Can you work these out from the model? Positions are in its coordinate system, mm. A direction names the side the tool comes from. Give positions to 0.01 mm unless a question says otherwise; leave off trailing zeros. Loops run counter-clockwise (first coordinate to the right, second up) from the corner with the lowest first, then second, coordinate; pieces in that order, holes last. Notation, with made-up numbers: (-11, 86) -> (28, 86) arc R18 cw to (28, 106) -> close; hole circle Ø3 at (-29, 49.25). An arc over 180 degrees is marked (long way). Return JSON: item names as keys, results as strings. Group by question number.
Q1. I need wall thicknesses on line 1 along Y through (x, z) = (-30, 0); line 2 along Y through (x, z) = (0, 11); line 3 along X through (y, z) = (-58, 2.5). Which ranges of each line are inside material? Lowest first, please. Write a range as [from, to].
Q2. Suppose I cut it at D-D, the plane y = -55. Please give me the cut outline in (x, z).
Q3. Will these pins go through, and if not, where does the flat tip stop? pin 1 (5 mm diameter, centred on x = -32, y = 23.5, fed in from -Z); pin 2 (1.5 mm diameter, centred on x = 6, z = 5.5, fed in from -Y); pin 3 (10 mm diameter, centred on y = 70.5, z = -10, fed in from -X); pin 4 (3 mm diameter, centred on y = 9, z = 6.5, fed in from +X).
Q4. Thinking about a two-plate mould opening in X: for faces 1 (the flat face through (19, -19, 4)), 2 (the cylindrical face through (41.53, -79.845, 0.056)), 3 (the cylindrical face through (-12.831, -46.555, 0.056)), which applies, pulls with the +X half, pulls with the -X half, needs draft (parallel to the pull), parting line crosses it, or undercut?
Q5. Suppose I cut it at A-A, the plane y = 0. Please give me the cut outline in (x, z).
Q6. Suppose I cut it at C-C, the plane x = 39.5. Please give me the cut outline in (y, z).
Q7. Which directions (+Z, -Z, +X, -X, +Y, -Y) give clear straight access to the entire face, cutting with the end or side of a thin tool? Please do faces 4 (the flat face through (0, -11, -22)), 5 (the cylindrical face through (23.846, 7.509, -12.874)), 6 (the cylindrical face through (23.846, 7.509, 13.126)).
Q8. Suppose I cut it at B-B, the plane x = 0. Please give me the cut outline in (y, z).
```python
from build123d import *

# Parameters (mm, degrees)
SKETCH_1_R          = 90
SKETCH_1_R_2        = 10.1
EXTRUDE_1_DEPTH     = 4
SKETCH_2_R          = 25
SKETCH_2_R_2        = 10.1
EXTRUDE_2_DEPTH     = 22
SKETCH_3_R          = 18
CUT_EXTRUDE_1_DEPTH = 30


with BuildPart() as part:
    # 草图1 → 凸台-拉伸1 (new, symmetric)
    with BuildSketch(Plane.XY):
        Circle(SKETCH_1_R)
        Circle(SKETCH_1_R_2, mode=Mode.SUBTRACT)
    extrude(amount=EXTRUDE_1_DEPTH, both=True)

    # 草图2 → 凸台-拉伸2 (add, symmetric)
    with BuildSketch(Plane.XY):
        Circle(SKETCH_2_R)
        Circle(SKETCH_2_R_2, mode=Mode.SUBTRACT)
    extrude(amount=EXTRUDE_2_DEPTH, both=True)

    # 草图3 → 切除-拉伸1 (cut, symmetric)
    with BuildSketch(Plane.XY):
        with Locations((60, 0)):
            Circle(SKETCH_3_R)
        with Locations((30, 51.961524227)):
            Circle(SKETCH_3_R)
        with Locations((-30, 51.961524227)):
            Circle(SKETCH_3_R)
        with Locations((-60, 0)):
            Circle(SKETCH_3_R)
        with Locations((-30, -51.961524227)):
            Circle(SKETCH_3_R)
        with Locations((30, -51.961524227)):
            Circle(SKETCH_3_R)
    extrude(amount=CUT_EXTRUDE_1_DEPTH, both=True, mode=Mode.SUBTRACT)


solid = part.part
```
Ans:
{
 "1": {"line 1": "y = [-84.85, -69.96], [-33.96, 33.96], [69.96, 84.85]", "line 2": "y = [-25, -10.1], [10.1, 25]", "line 3": "x = [-68.82, -46.96], [-13.04, 13.04], [46.96, 68.82]"},
 "2": {"outline": "(-71.24, -4) -> (-47.74, -4) -> (-47.74, 4) -> (-71.24, 4) -> close; (-12.26, -4) -> (12.26, -4) -> (12.26, 4) -> (-12.26, 4) -> close; (47.74, -4) -> (71.24, -4) -> (71.24, 4) -> (47.74, 4) -> close"},
 "3": {"pin 1": "stops at z = -4", "pin 2": "stops at y = -24.44", "pin 3": "passes through", "pin 4": "stops at x = 23.85"},
 "4": {"face 1": "needs draft", "face 2": "parting line crosses it", "face 3": "undercut"},
 "5": {"outline": "(-90, -4) -> (-78, -4) -> (-78, 4) -> (-90, 4) -> close; (-42, -4) -> (-25, -4) -> (-25, -22) -> (-10.1, -22) -> (-10.1, 22) -> (-25, 22) -> (-25, 4) -> (-42, 4) -> close; (10.1, -22) -> (25, -22) -> (25, -4) -> (42, -4) -> (42, 4) -> (25, 4) -> (25, 22) -> (10.1, 22) -> close; (78, -4) -> (90, -4) -> (90, 4) -> (78, 4) -> close"},
 "6": {"outline": "(-80.87, -4) -> (-67.25, -4) -> (-67.25, 4) -> (-80.87, 4) -> close; (-36.67, -4) -> (36.67, -4) -> (36.67, 4) -> (-36.67, 4) -> close; (67.25, -4) -> (80.87, -4) -> (80.87, 4) -> (67.25, 4) -> close"},
 "7": {"face 4": "-Z, +X, -X, +Y, -Y", "face 5": "-Z", "face 6": "+Z"},
 "8": {"outline": "(-90, -4) -> (-25, -4) -> (-25, -22) -> (-10.1, -22) -> (-10.1, 22) -> (-25, 22) -> (-25, 4) -> (-90, 4) -> close; (10.1, -22) -> (25, -22) -> (25, -4) -> (90, -4) -> (90, 4) -> (25, 4) -> (25, 22) -> (10.1, 22) -> close"}
}
